from build123d import *

# Parameters (mm, degrees)
SKETCH1_R           = 3.5
SKETCH1_R_2         = 4
BOSS_EXTRUDE1_DEPTH = 5.4


with BuildPart() as part:
    # Sketch1 → Boss-Extrude1 (new body)
    with BuildSketch(Plane.XY):
        with BuildLine():
            Line((-8.997274893, 37.552834761), (-7.747259547, -13.231665239))
            ThreePointArc((-7.747259547, -13.231665239), (1.471475273, -22.007480205), (10.247290239, -12.788745384))
            Line((10.247290239, -12.788745384), (9.197993195, 29.841151848))
            ThreePointArc((9.197993195, 29.841151848), (9.816337009, 32.376738458), (11.627190957, 34.256194898))
            Line((11.627190957, 34.256194898), (22.36781842, 40.697064727))
            ThreePointArc((22.36781842, 40.697064727), (25.457229961, 53.042113109), (13.11218158, 56.13152465))
            Line((13.11218158, 56.13152465), (-4.628608734, 45.492842556))
            ThreePointArc((-4.628608734, 45.492842556), (-7.885246166, 42.11283049), (-8.997274893, 37.552834761))
        make_face()
        with Locations(Location((0, 37.774294688, 0), (0, 0, 180))):
            Circle(SKETCH1_R, mode=Mode.SUBTRACT)
        with Locations(Location((1.250015346, -13.010205312, 0), (0, 0, 180))):
            Circle(SKETCH1_R, mode=Mode.SUBTRACT)
        with Locations(Location((17.74, 48.414294688, 0), (0, 0, 180))):
            Circle(SKETCH1_R_2, mode=Mode.SUBTRACT)
    extrude(amount=BOSS_EXTRUDE1_DEPTH)


solid = part.part
Build history of the part. All positions in model axes, mm. A direction names the side the tool comes from. Coordinates: 2 decimals unless noted, no trailing zeros. Order: outer loops, then holes, each group sorted by start corner. A loop starts at its lowest first (then second) coordinate and runs counter-clockwise, first axis right, second up. Notation, with made-up numbers: M 15.5,-31.75 L 24.5,-31.75 A18 cw 24.5,-25.75 Z; hole C 60.5,33.25 d10. An arc over 180 degrees is marked long. One line per question, with ' | ' between items. Start each with the question number.
Q1. Probe L1, parallel to Y at x = 0, z = 2.8; L2, parallel to Y at x = 16, z = 4.9; L3, parallel to Y at x = 17.74, z = 3.55. List the from-to ranges inside material, lowest first. Write a range as from..to.
Q2. Saw through at C-C (z = 0.95). List the corners of the cut face in (x, y), then the cut area to 3 significant figures.
Q3. Saw through at B-B (x = 17.74). List the corners of the cut face in (y, z).
Q4. Flat gauge pins, fed straight in: pin 1 Ø5 at (x, y) = (17.74, 48.41) entering from +Z; pin 2 Ø1 at (y, z) = (39.5, 2) entering from +X; pin 3 Ø1.5 at (x, z) = (10, 3) entering from +Y (3 decimals); pin 4 Ø1 at (x, z) = (9.5, 2) entering from +Y. Where does each tip first touch, or does it go through?
Q5. Saw through at A-A (y = -10.5). List the corners of the cut face in (x, z), then the cut area to 3 significant figures.
Q6. 3-axis set-ups, long thin cutter, end or side, ignore diameter. For faces 1 (the face through (4.37, 50.89, 2.66)), 2 (the face through (9.799, 32.344, 2.662)): which of +Z, -Z, +X, -X, +Y, -Y reach the whole face in a straight line?
Q7. Saw through at D-D (x = 0). List the corners of the cut face in (y, z).
Q8. Two-plate mould, pull along X, no slides. Class faces 3 (the face through (5, 18, 0)), 4 (the face through (15.89, 51.96, 2.66)), 5 (the face through (-7.853, 42.171, 2.662)): +X half, -X half, draft (parallel to the pull), parting line (faces both ways), or undercut.
Check values:
1) L1: y = -21.92..-16.28, -9.74..34.27, 41.27..48.27 | L2: y = 36.88..44.81, 52.02..57.24 | L3: y = 37.92..44.41, 52.41..57.41
2) outline: M -9,37.55 L -7.75,-13.23 A9 ccw 10.25,-12.79 L 9.2,29.84 A5 cw 11.63,34.26 L 22.37,40.7 A9 ccw 13.11,56.13 L -4.63,45.49 A9 ccw Z; hole C 0,37.77 d7; hole C 1.25,-13.01 d7; hole C 17.74,48.41 d8 | area: 1,410 mm2
3) outline: M 37.92,0 L 44.41,0 L 44.41,5.4 L 37.92,5.4 Z; M 52.41,0 L 57.41,0 L 57.41,5.4 L 52.41,5.4 Z
4) pin 1: passes through | pin 2: stops at x = 21.21 | pin 3: stops at y = 54.715 | pin 4: stops at y = 54.27
5) outline: M -7.81,0 L -1.19,0 L -1.19,5.4 L -7.81,5.4 Z; M 3.69,0 L 10.19,0 L 10.19,5.4 L 3.69,5.4 Z | area: 70.9 mm2
6) face 1: +Z, -Z, -X, +Y | face 2: +Z, -Z, +X
7) outline: M -21.92,0 L -16.28,0 L -16.28,5.4 L -21.92,5.4 Z; M -9.74,0 L 34.27,0 L 34.27,5.4 L -9.74,5.4 Z; M 41.27,0 L 48.27,0 L 48.27,5.4 L 41.27,5.4 Z
8) face 3: draft | face 4: undercut | face 5: -X half
